Job drawing, mm, ordinate dimensions from the low corner. One solid piece. Give positions to 0.01 mm unless a question says otherwise; leave off trailing zeros. Write each loop counter-clockwise with the first axis right and the second up, starting at its lowest first coordinate (ties: lowest second). Pieces come first, ordered by that corner, then holes. Notation, with made-up numbers: M 81,-15.75 L 91,-15.75 A28 cw 91,16.25 Z; hole C 4,52.5 d11. An arc over 180 degrees is marked long. Answer as CSV lines item,"result". Start each with the question number.
Item 1: Band-saw the part on B-B, the plane z = 40. List the corners of the cut face in (x, y), then the cut area to 3 significant figures.
Item 2: Wall check: L1, parallel to X at y = 0.6, z = 40; L2, parallel to X at y = 1.45, z = 39.5 (1 decimal); L3, parallel to X at y = 0.6, z = 73 (1 decimal). Give the ranges that are in metal, low to high. Write a range as from..to.
Item 3: Band-saw the part on A-A, the plane x = 40. List the corners of the cut face in (y, z).
Item 4: Band-saw the part on D-D, the plane z = 21. List the corners of the cut face in (x, y), then the cut area to 3 significant figures.
Item 5: Band-saw the part on C-C, the plane y = 1.3. List the corners of the cut face in (x, z), then the cut area to 3 significant figures.
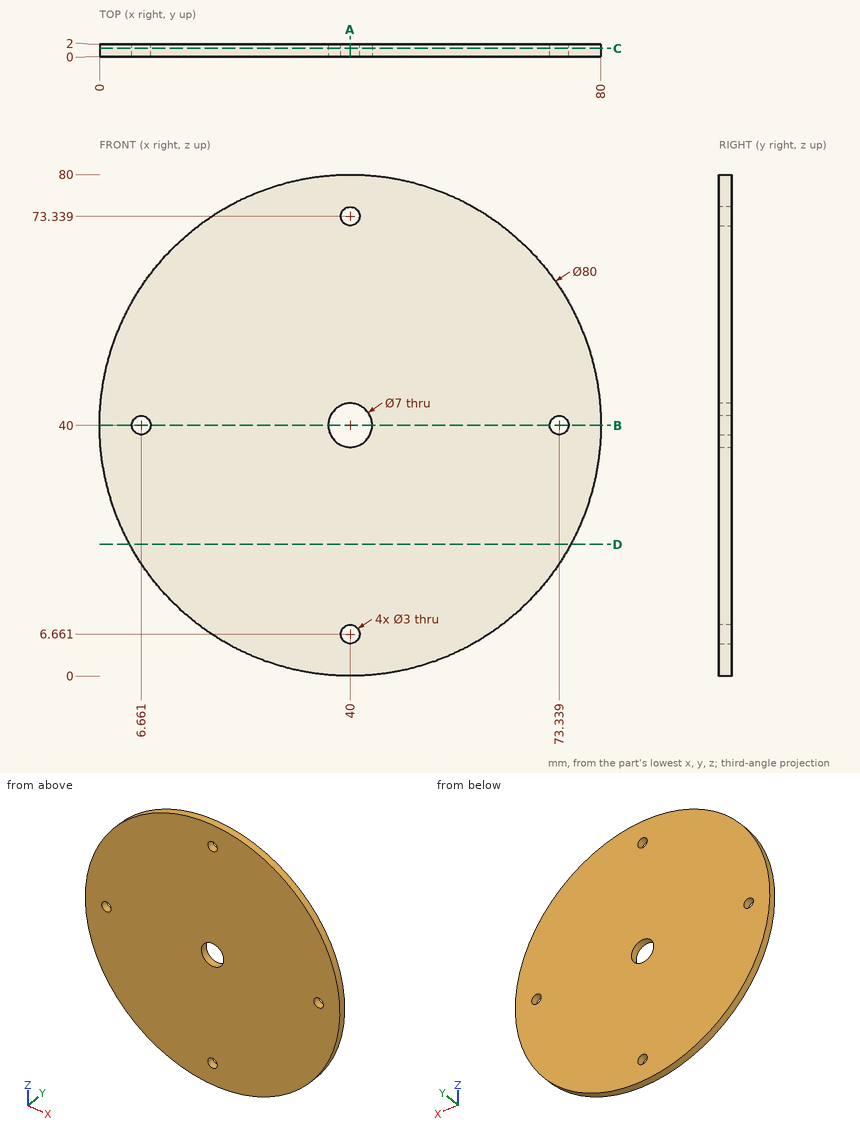
Output:
1,outline,"M 0,0 L 5.16,0 L 5.16,2 L 0,2 Z; M 8.16,0 L 36.5,0 L 36.5,2 L 8.16,2 Z; M 43.5,0 L 71.84,0 L 71.84,2 L 43.5,2 Z; M 74.84,0 L 80,0 L 80,2 L 74.84,2 Z"
1,area,"134 mm²"
2,L1,"0..5.16, 8.16..36.5, 43.5..71.84, 74.84..80"
2,L2,"0..5.2, 8.1..36.5, 43.5..71.9, 74.8..80"
2,L3,"17.4..38.5, 41.5..62.6"
3,outline,"M 0,0 L 2,0 L 2,5.16 L 0,5.16 Z; M 0,8.16 L 2,8.16 L 2,36.5 L 0,36.5 Z; M 0,43.5 L 2,43.5 L 2,71.84 L 0,71.84 Z; M 0,74.84 L 2,74.84 L 2,80 L 0,80 Z"
4,outline,"M 4.8,0 L 75.2,0 L 75.2,2 L 4.8,2 Z"
4,area,"141 mm²"
5,outline,"C 40,40 d80; hole C 6.66,40 d3; hole C 40,40 d7; hole C 40,6.66 d3; hole C 40,73.34 d3; hole C 73.34,40 d3"
5,area,"4,960 mm²"
